from build123d import *

# Parameters (mm, degrees)
SKETCH_1_R      = 31.5
SKETCH_1_R_2    = 25.25
EXTRUDE_1_DEPTH = 20
CHAMFER_1_SIZE  = 0.5


with BuildPart() as part:
    # 草图1 → 凸台-拉伸1 (new body)
    with BuildSketch(Plane.XY):
        Circle(SKETCH_1_R)
        Circle(SKETCH_1_R_2, mode=Mode.SUBTRACT)
    extrude(amount=EXTRUDE_1_DEPTH)

    # 倒角1
    chamfer_1_edges = [part.edges().sort_by_distance(p)[0] for p in [
        (-31.5, 0, 0),
        (-31.5, 0, 20),
        (-25.25, 0, 0),
        (-25.25, 0, 20),
    ]]
    chamfer(chamfer_1_edges, length=CHAMFER_1_SIZE)


solid = part.part
Check sheet for the modelled part. Datum: model origin and axes. Units: mm. Round coordinates to 2 decimals unless told otherwise and drop trailing zeros. Order: outer loops, then holes, each group sorted by start corner. A loop starts at its lowest first (then second) coordinate and runs counter-clockwise, first axis right, second up. Notation, with made-up numbers: M 15.25,81.5 L 23.25,81.5 A17 ccw 23.25,109.5 Z; hole C -33.75,41.25 d10. An arc over 180 degrees is marked long. One line per item, written item: value. Start each with the question number.
1. Scan lines: line 1 along X through (y, z) = (-20.5, 1.25); line 2 along X through (y, z) = (18, 8.75); line 3 along Y through (x, z) = (0, 11). Record each from-to range of solid material in increasing order.
2. Release check for a two-part mould opening along X. For faces 1 (the cylindrical face through (-5.47, -24.65, 9.87)), 2 (the flat face through (-12, 23, 0)), 3 (the cylindrical face through (-4.101, 31.232, 9.867)) record: released by +X, released by -X, zero draft, split by the parting line, or undercut.
3. Section check A-A on y = 0. Enter the section's corners in (x, z), and give its area (3 significant figures).
4. Gauge pin test, flat ends, axial feed: P1, Ø8, axis at x = 10.5, z = 11, coming from the -Y side; P2, Ø5, axis at x = -8.5, z = 5, coming from the +Y side; P3, Ø3, axis at x = -22.5, y = 13.5, coming from the -Z side; P4, Ø2, axis at y = 18, z = 10, coming from the +X side. Record the tip position at first contact, or that the pin passes through.
5. Section check C-C on z = 15.75. Enter the section's corners in (x, y), and give its area (3 significant figures).
Results found:
1. line 1: -23.92 to -14.74, 14.74 to 23.92
1. line 2: -25.85 to -17.71, 17.71 to 25.85
1. line 3: -31.5 to -25.25, 25.25 to 31.5
2. face 1: undercut
2. face 2: zero draft
2. face 3: split by the parting line
3. outline: M -31.5,0.5 L -31,0 L -25.75,0 L -25.25,0.5 L -25.25,19.5 L -25.75,20 L -31,20 L -31.5,19.5 Z; M 25.25,0.5 L 25.75,0 L 31,0 L 31.5,0.5 L 31.5,19.5 L 31,20 L 25.75,20 L 25.25,19.5 Z
3. area: 249 mm^2
4. P1: y = -30.82
4. P2: y = 30.92
4. P3: z = 0
4. P4: x = 26.52
5. outline: C 0,0 d63; hole C 0,0 d50.5
5. area: 1,110 mm^2
